from build123d import *

# Parameters (mm, degrees)
BOSS_EXTRUDE1_DEPTH = 6
SKETCH3_W           = 6
SKETCH3_H           = 60
CUT_EXTRUDE1_DEPTH  = 10
CUT_EXTRUDE2_DEPTH  = 187.01085661


with BuildPart() as part:
    # Sketch1 → Boss-Extrude1 (new body)
    with BuildSketch(Plane.XY):
        Polygon((127.020625139, -33.445286794), (107.020625139, -33.445286794), (107.020625139, 70.514713206), (172.022422952, 70.514713206), (172.022422952, -33.445286794), (152.022422952, -33.445286794), (152.022422952, -23.465104548), (127.020625139, -23.465104548), align=None)
    extrude(amount=BOSS_EXTRUDE1_DEPTH)

    # Sketch3 → Cut-Extrude1 (cut)
    with BuildSketch(Plane(origin=(0, 0, 0), x_dir=(-1, 0, 0), z_dir=(0, 0, -1))):
        with Locations((-139.522422952, -14.485286794)):
            Rectangle(SKETCH3_W, SKETCH3_H)
    extrude(amount=-CUT_EXTRUDE1_DEPTH, mode=Mode.SUBTRACT)

    # Sketch4 → Cut-Extrude2 (cut, through all)
    with BuildSketch(Plane.XY.offset(6)):
        Polygon((124.522422952, -36.580409203), (107.020625139, -36.580409203), (107.020625139, 70.514713206), (120.512520278, 70.514713206), (126.522422952, 70.514713206), (126.522422952, 10.514713206), (124.522422952, 10.514713206), align=None)
    extrude(amount=-CUT_EXTRUDE2_DEPTH, mode=Mode.SUBTRACT)


solid = part.part
Input: part model. Units: mm. Frame: model coordinates. A direction names the side the tool comes from. Give positions to 0.01 mm unless a question says otherwise; leave off trailing zeros. Write each loop counter-clockwise with the first axis right and the second up, starting at its lowest first coordinate (ties: lowest second). Pieces come first, ordered by that corner, then holes. Notation, with made-up numbers: M -23,74 L 16,74 A9 cw 16,80 Z; hole C 70,17.5 d3. An arc over 180 degrees is marked long. Write item = value, one per line. Start each with the question number.
1) Cut plane D-D on x = 134. Return the cut outline in (y, z).
2) Cut plane C-C on y = -10.5. Return the cut outline in (x, z), then the cut area to 3 significant figures.
3) Cut plane B-B on z = 2.95. Return the cut outline in (x, y).
4) Material intervals for line 1 along X through (y, z) = (-22, 0.3); line 2 along X through (y, z) = (12.5, 4.9); line 3 along Y through (x, z) = (131.5, 4.55), sorted ascending. Write a range as [from, to].
5) Reachability of faces 1 (the flat face through (152.022, -29, 3)), 2 (the flat face through (172.022, 19, 3)), 3 (the flat face through (126, 10.515, 3)) from +Z, -Z, +X, -X, +Y, -Y: full face, straight path, thin tool, end or side. Return the list, or none.
6) Cut plane A-A on y = 14.5. Return the cut outline in (x, z).
7) Draft query along X for faces 4 (the flat face through (126.522, 41, 3)), 5 (the flat face through (132, -23.465, 3)), 6 (the flat face through (126, -33.445, 3)). Return one class per face: +X half, -X half, draft (parallel to the pull), parting line (faces both ways), or undercut.
8) First-contact query: pin 1 Ø2 at (x, z) = (125, 2) entering from +Y. Flat tip, straight axial feed; report the tip coordinate or a pass-through.
Solved:
q1.outline = M -23.47,0 L 70.51,0 L 70.51,6 L -23.47,6 Z
q2.outline = M 124.52,0 L 136.52,0 L 136.52,6 L 124.52,6 Z; M 142.52,0 L 172.02,0 L 172.02,6 L 142.52,6 Z
q2.area = 249 mm2
q3.outline = M 124.52,-33.45 L 127.02,-33.45 L 127.02,-23.47 L 136.52,-23.47 L 136.52,15.51 L 142.52,15.51 L 142.52,-23.47 L 152.02,-23.47 L 152.02,-33.45 L 172.02,-33.45 L 172.02,70.51 L 126.52,70.51 L 126.52,10.51 L 124.52,10.51 Z
q4.line_1 = [124.52, 136.52], [142.52, 172.02]
q4.line_2 = [126.52, 136.52], [142.52, 172.02]
q4.line_3 = [-23.47, 70.51]
q5.face_1 = +Z, -Z, -Y
q5.face_2 = +Z, -Z, +X, +Y, -Y
q5.face_3 = +Z, -Z, -X, +Y
q6.outline = M 126.52,0 L 136.52,0 L 136.52,6 L 126.52,6 Z; M 142.52,0 L 172.02,0 L 172.02,6 L 142.52,6 Z
q7.face_4 = -X half
q7.face_5 = undercut
q7.face_6 = draft
q8.pin_1 = 10.51
